Source: three-view drawing plus pictorial views. Frame: mm from the lowest corner of the part. Give positions to 0.01 mm unless a question says otherwise; leave off trailing zeros. Loops run counter-clockwise (first coordinate to the right, second up) from the corner with the lowest first, then second, coordinate; pieces in that order, holes last. Notation, with made-up numbers: (75.5, 9) - (106.5, 9) arc R18 cw to (106.5, 31) - close; hole circle Ø1 at (9.5, 75.25). An arc over 180 degrees is marked (long way). One line per item, written item: value.
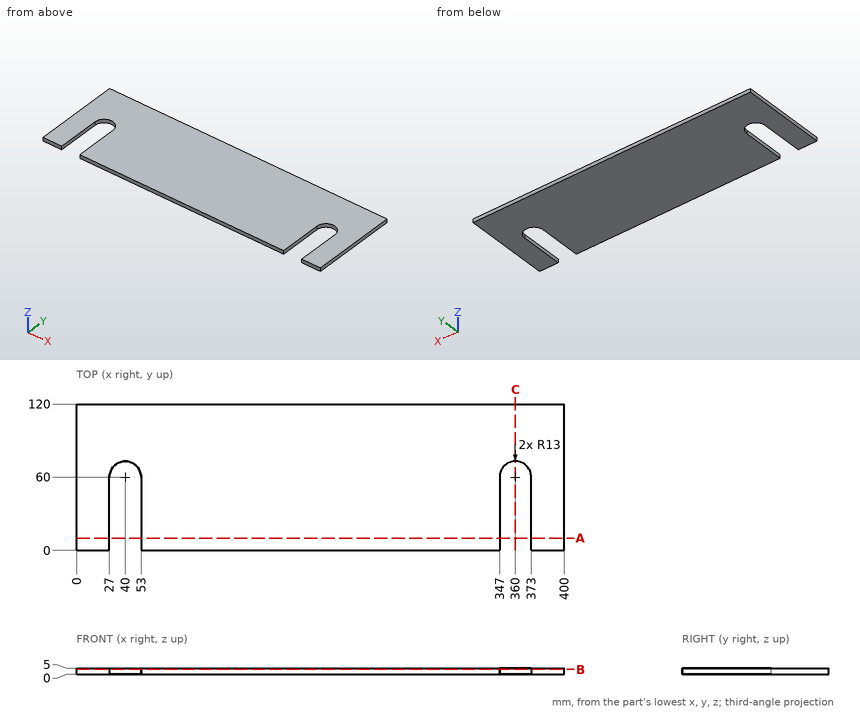
Item 1: Section B-B, the plane z = 4.2. Output: boundary loops of the cut face in (x, y).
Verdict:
outline: (0, 0) - (27, 0) - (27, 60) arc R13 cw to (53, 60) - (53, 0) - (347, 0) - (347, 60) arc R13 cw to (373, 60) - (373, 0) - (400, 0) - (400, 120) - (0, 120) - close
Item 2: Pin query (flat end, axial travel): P1, Ø1.5, axis at y = 24, z = 1.5, coming from the -X side. Return the tip coordinate at first contact, or that it passes through.
Verdict:
P1: stops at x = 0
Item 3: Section A-A, the plane y = 10. Output: boundary loops of the cut face in (x, z), and give its area (3 significant figures).
Verdict:
outline: (0, 0) - (27, 0) - (27, 5) - (0, 5) - close; (53, 0) - (347, 0) - (347, 5) - (53, 5) - close; (373, 0) - (400, 0) - (400, 5) - (373, 5) - close
area: 1,740 mm^2
Item 4: Material intervals for L1, parallel to X at y = 11.5, z = 3.95; L2, parallel to Y at x = 51.5, z = 0.6; L3, parallel to Y at x = 365, z = 4.5, sorted ascending.
Verdict:
L1: x = 0 to 27, 53 to 347, 373 to 400
L2: y = 66.06 to 120
L3: y = 72 to 120
Item 5: Section C-C, the plane x = 360. Output: boundary loops of the cut face in (y, z), and give its area (3 significant figures).
Verdict:
outline: (73, 0) - (120, 0) - (120, 5) - (73, 5) - close
area: 235 mm^2
